Input: dimensioned drawing with shaded views. Units: mm. Origin: part minimum x, y, z. Round coordinates to 2 decimals unless told otherwise and drop trailing zeros. Loops run counter-clockwise (first coordinate to the right, second up) from the corner with the lowest first, then second, coordinate; pieces in that order, holes last. Notation, with made-up numbers: M 46,-7.75 L 74,-7.75 A8 cw 74,6.25 Z; hole C 50.5,-32 d5. An arc over 180 degrees is marked long. One line per item, written item: value.
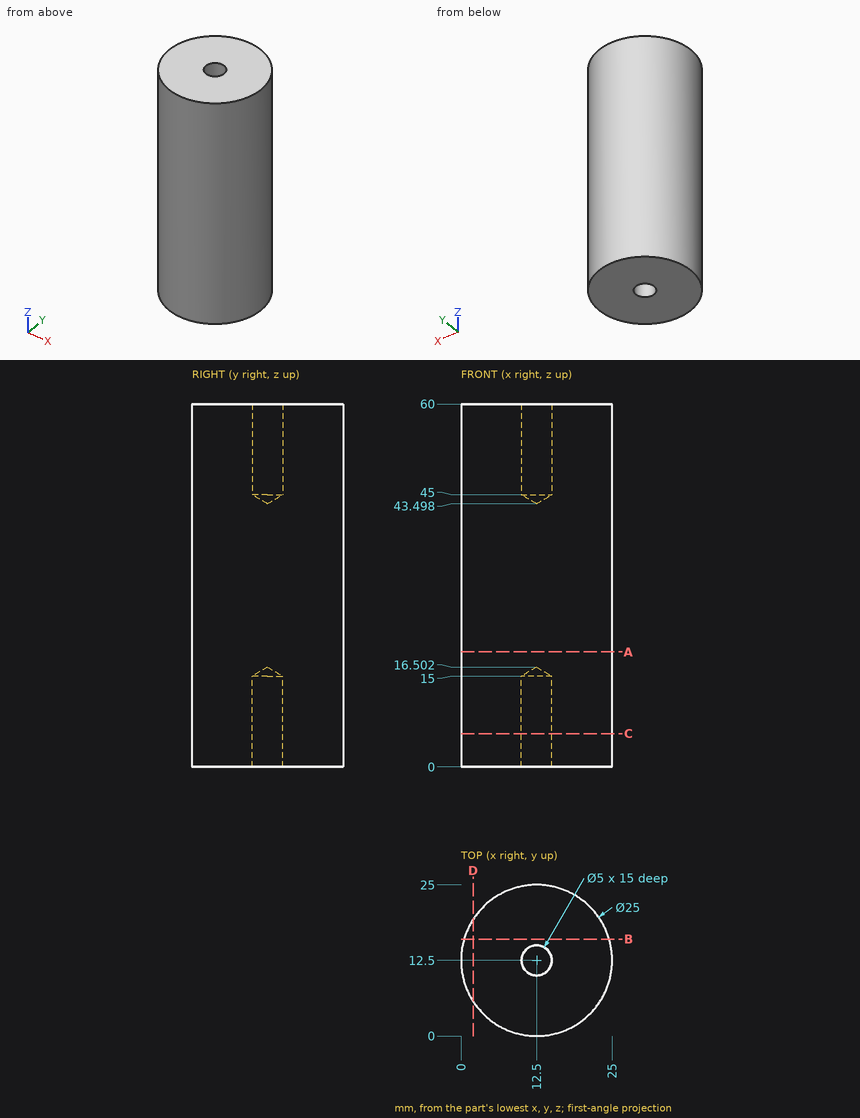
1. Section query C-C (z = 5.5). Return the cut outline in (x, y).
Report:
outline: C 12.5,12.5 d25; hole C 12.5,12.5 d5
2. Section query B-B (y = 16). Return the cut outline in (x, z), and give its area (3 significant figures).
Report:
outline: M 0.5,0 L 24.5,0 L 24.5,60 L 0.5,60 Z
area: 1,440 mm2
3. Section query A-A (z = 19). Return the cut outline in (x, y), and give its area (3 significant figures).
Report:
outline: C 12.5,12.5 d25
area: 491 mm2
4. Section query D-D (x = 2). Return the cut outline in (y, z).
Report:
outline: M 5.72,0 L 19.28,0 L 19.28,60 L 5.72,60 Z
5. Pin query (flat end, axial travel): pin 1 (12 mm diameter, centred on x = 20, z = 14, fed in from -Y); pin 2 (3 mm diameter, centred on x = 12.5, y = 12.5, fed in from +Z); pin 3 (6 mm diameter, centred on y = 3.5, z = 44, fed in from -X). Return the tip coordinate at first contact, or that it passes through.
Report:
pin 1: stops at y = 0.09
pin 2: stops at z = 44.4
pin 3: stops at x = 1.53
6. Ray query, line 1 (Y direction, x = 12.5, z = 48); line 2 (X direction, y = 13.25, z = 57.5) (1 decimal); line 3 (X direction, y = 12.25, z = 39.5). Return the intervals inside material, ascending. Write a range as [from, to].
Report:
line 1: y = [0, 10], [15, 25]
line 2: x = [0, 10.1], [14.9, 25]
line 3: x = [0, 25]
